Check sheet for the drawn part. Datum: minimum x, y, z corner. Units: mm. Round coordinates to 2 decimals unless told otherwise and drop trailing zeros. Write each loop counter-clockwise with the first axis right and the second up, starting at its lowest first coordinate (ties: lowest second). Pieces come first, ordered by that corner, then holes. Notation, with made-up numbers: M -23.75,3 L 16.25,3 A24 ccw 16.25,17 Z; hole C -28.75,-12.5 d9. An arc over 180 degrees is marked long. Use a Markdown table: item, result.
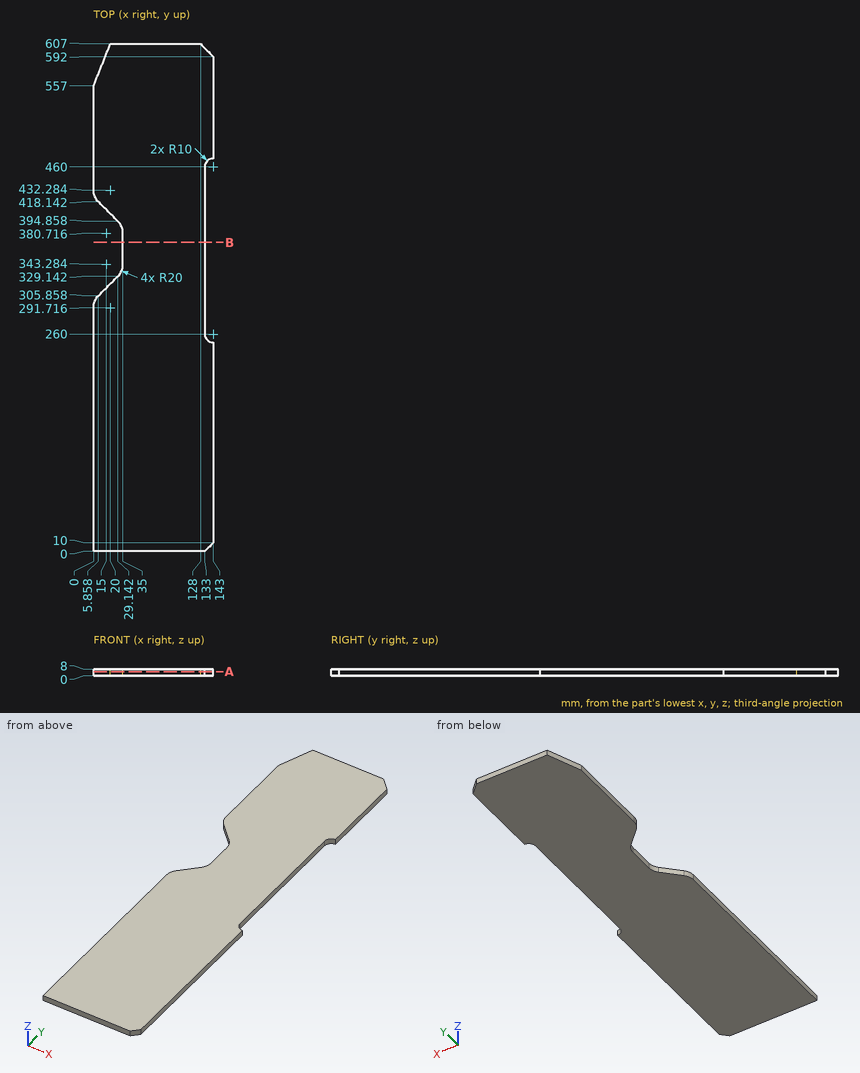
Item 1: Material ranges on line 1 along X through (y, z) = (285, 3); line 2 along X through (y, z) = (348.5, 4); line 3 along Y through (x, z) = (131.5, 5), recorded low to high. Write a range as from..to.
Outcome:
| item | result |
|---|---|
| line 1 | x = 0..133 |
| line 2 | x = 35..133 |
| line 3 | y = 0..603.5 |
Item 2: Cross-section at B-B, the plane y = 369.5. Record the cut outline in (x, z), and give its area (3 significant figures).
Outcome:
| item | result |
|---|---|
| outline | M 35,0 L 133,0 L 133,8 L 35,8 Z |
| area | 784 mm2 |
Item 3: Cross-section at A-A, the plane z = 5.25. Record the cut outline in (x, y), and give its area (3 significant figures).
Outcome:
| item | result |
|---|---|
| outline | M 0,0 L 133,0 L 143,10 L 143,250 A10 cw 133,260 L 133,460 A10 cw 143,470 L 143,592 L 128,607 L 20,607 L 0,557 L 0,432.28 A20 ccw 5.86,418.14 L 29.14,394.86 A20 cw 35,380.72 L 35,343.28 A20 cw 29.14,329.14 L 5.86,305.86 A20 ccw 0,291.72 Z |
| area | 80,900 mm2 |
Item 4: Go/stop test with a flat-tipped pin: pin 1 (4 mm diameter, centred on y = 363.5, z = 4, fed in from -X). Record where the tip stops, or that it passes through.
Outcome:
| item | result |
|---|---|
| pin 1 | stops at x = 35 |
